```python
from build123d import *

# Parameters (mm, degrees)
SKETCH1_W                                          = 55
SKETCH1_H                                          = 24
BOSS_EXTRUDE1_DEPTH                                = 10
HOLE_WIZARD_3_D                                    = 4.5
HOLE_WIZARD_3_DEPTH                                = 12.4
HOLE_WIZARD_3_CBORE_D                              = 8
HOLE_WIZARD_3_CBORE_DEPTH                          = 4.6
HOLE_WIZARD_3_TIP                                  = 1.351936393
SKETCH6_W                                          = 5
SKETCH6_H                                          = 24
BOSS_EXTRUDE2_DEPTH                                = 10
CHAMFER1_SIZE                                      = 3
CHAMFER2_SIZE                                      = 0.5
HOLE_SIZE_BASED_ON_SOCKET_HEAD_CAP_SCR_D           = 5.5
HOLE_SIZE_BASED_ON_SOCKET_HEAD_CAP_SCR_DEPTH       = 12.4
HOLE_SIZE_BASED_ON_SOCKET_HEAD_CAP_SCR_CBORE_D     = 10
HOLE_SIZE_BASED_ON_SOCKET_HEAD_CAP_SCR_CBORE_DEPTH = 5.7
HOLE_SIZE_BASED_ON_SOCKET_HEAD_CAP_SCR_TIP         = 1.652366702
M5_TAPPED_HOLE1_D                                  = 4.2


with BuildPart() as part:
    # Sketch1 → Boss-Extrude1 (new body)
    with BuildSketch(Plane(origin=(0, 0, 0), x_dir=(1, 0, 0), z_dir=(0, 1, 0))):
        with Locations((-1.42708605, -3.163732927)):
            Rectangle(SKETCH1_W, SKETCH1_H)
    extrude(amount=BOSS_EXTRUDE1_DEPTH)

    # 打孔尺寸(%根据)内六角圆柱头螺钉的类型3
    with Locations(Plane(origin=(0, 0, 0), x_dir=(-1, 0, 0), z_dir=(0, -1, 0))):
        with Locations((23.92708605, -3.163732927), (-1.07291395, -3.163732927)):
            CounterBoreHole(HOLE_WIZARD_3_D / 2, HOLE_WIZARD_3_CBORE_D / 2, HOLE_WIZARD_3_CBORE_DEPTH, depth=HOLE_WIZARD_3_DEPTH)
            with Locations((0, 0, -(HOLE_WIZARD_3_DEPTH + HOLE_WIZARD_3_TIP / 2))):  # 118° drill point
                Cone(0, HOLE_WIZARD_3_D / 2, HOLE_WIZARD_3_TIP, mode=Mode.SUBTRACT)

    # Sketch6 → Boss-Extrude2 (add)
    with BuildSketch(Plane.XZ):
        with Locations((28.57291395, 3.163732927)):
            Rectangle(SKETCH6_W, SKETCH6_H)
    extrude(amount=-BOSS_EXTRUDE2_DEPTH)

    # Chamfer1
    chamfer1_edges = [part.edges().sort_by_distance(p)[0] for p in [
        (31.07291395, 5, 15.163732927),
        (31.07291395, 5, -8.836267073),
        (-28.92708605, 5, -8.836267073),
        (-28.92708605, 5, 15.163732927),
    ]]
    chamfer(chamfer1_edges, length=CHAMFER1_SIZE)

    # Chamfer2
    chamfer2_edges = [part.edges().sort_by_distance(p)[0] for p in [
        (1.07291395, 0, -8.836267073),
        (1.07291395, 10, -8.836267073),
        (-28.92708605, 0, 3.163732927),
        (31.07291395, 0, 3.163732927),
        (1.07291395, 0, 15.163732927),
        (31.07291395, 10, 3.163732927),
        (-28.92708605, 10, 3.163732927),
        (1.07291395, 10, 15.163732927),
    ]]
    chamfer(chamfer2_edges, length=CHAMFER2_SIZE)

    # Hole Size _Based On_ Socket Head Cap Scr
    with Locations(Plane(origin=(0, 0, 0), x_dir=(-1, 0, 0), z_dir=(0, -1, 0))):
        with Locations((-23.07291395, -3.163732927)):
            CounterBoreHole(HOLE_SIZE_BASED_ON_SOCKET_HEAD_CAP_SCR_D / 2, HOLE_SIZE_BASED_ON_SOCKET_HEAD_CAP_SCR_CBORE_D / 2, HOLE_SIZE_BASED_ON_SOCKET_HEAD_CAP_SCR_CBORE_DEPTH, depth=HOLE_SIZE_BASED_ON_SOCKET_HEAD_CAP_SCR_DEPTH)
            with Locations((0, 0, -(HOLE_SIZE_BASED_ON_SOCKET_HEAD_CAP_SCR_DEPTH + HOLE_SIZE_BASED_ON_SOCKET_HEAD_CAP_SCR_TIP / 2))):  # 118° drill point
                Cone(0, HOLE_SIZE_BASED_ON_SOCKET_HEAD_CAP_SCR_D / 2, HOLE_SIZE_BASED_ON_SOCKET_HEAD_CAP_SCR_TIP, mode=Mode.SUBTRACT)

    # M5 Tapped Hole1 (through all)
    with Locations(Plane(origin=(0, 10, 0), x_dir=(1, 0, 0), z_dir=(0, 1, 0))):
        with Locations((-11.92708605, -3.163732927), (13.07291395, -3.163732927)):
            Hole(M5_TAPPED_HOLE1_D / 2)


solid = part.part
```
Source: CAD feature listing. Evaluate the final solid. Frame: model axes, mm. A direction names the side the tool comes from. Coordinates: 2 decimals unless noted, no trailing zeros. Loops run counter-clockwise (first coordinate to the right, second up) from the corner with the lowest first, then second, coordinate; pieces in that order, holes last. Notation, with made-up numbers: (71, -12) -> (76, -12) arc R24 ccw to (76, 2) -> close; hole circle Ø2 at (-17.5, 16). An arc over 180 degrees is marked (long way). One line per item, written item: value. Start each with the question number.
Q1. Section query C-C, the plane x = -22.5. Return the cut outline in (y, z).
Q2. Contact query for flat-ended pins moving along their axis: P1, Ø7, axis at x = 1.07, z = 3.16, coming from the -Y side; P2, Ø6.5, axis at x = -23, z = 4.5, coming from the -Y side; P3, Ø9, axis at x = 23.07, z = 3.16, coming from the -Y side. Output: stop coordinate, or through.
Q3. Section query A-A, the plane x = 0.5. Return the cut outline in (y, z).
Q4. Section query D-D, the plane z = 4. Give the number of separate pieces and of enclosed holes in the cut face, and give its area (3 significant figures).
Q5. Set-up query: faces 5 (the face through (20.9, 5.7, 5.3)), 6 (the face through (0.78, 7.338, 0.933)). Return all of +Z, -Z, +X, -X, +Y, -Y with unobstructed straight access to the full face (end or side cutting, diameter ignored); none if empty.
Q6. Section query B-B, the plane y = 8.5. Return the cut outline in (x, z), and give its area (3 significant figures).
Q7. Mould query, pull axis Z, two halves, no side actions, for faces 1 (the face through (-27.448, 4.93, -7.315)), 2 (the face through (25.696, 7.88, 2.338)), 3 (the face through (5.07, 2.27, 2.99)), 4 (the face through (-27.45, 4.93, 13.64)). Classes: pulls with the +Z half, pulls with the -Z half, needs draft (parallel to the pull), parting line crosses it, or undercut.
Q8. Line query: line 1 along X through (y, z) = (4.5, -0.25); line 2 along X through (y, z) = (6.75, 4); line 3 along Z through (x, y) = (12, 3.5). Output: solid intervals per line, ascending.
Results:
1. outline: (0, -8.34) -> (0.5, -8.84) -> (9.5, -8.84) -> (10, -8.34) -> (10, 1.42) -> (4.6, 1.42) -> (4.6, -0.57) -> (0, -0.57) -> close; (0, 6.9) -> (4.6, 6.9) -> (4.6, 4.9) -> (10, 4.9) -> (10, 14.66) -> (9.5, 15.16) -> (0.5, 15.16) -> (0, 14.66) -> close
2. P1: y = 4.6
2. P2: y = 0
2. P3: y = 5.7
3. outline: (0, -8.34) -> (0.5, -8.84) -> (9.5, -8.84) -> (10, -8.34) -> (10, 0.99) -> (4.6, 0.99) -> (4.6, -0.8) -> (0, -0.8) -> close; (0, 7.12) -> (4.6, 7.12) -> (4.6, 5.34) -> (10, 5.34) -> (10, 14.66) -> (9.5, 15.16) -> (0.5, 15.16) -> (0, 14.66) -> close
4. separate pieces: 6
4. enclosed holes: 0
4. area: 327 mm^2
5. face 5: -Y
5. face 6: +Y, -Y
6. outline: (-28.93, -5.84) -> (-25.93, -8.84) -> (28.07, -8.84) -> (31.07, -5.84) -> (31.07, 12.16) -> (28.07, 15.16) -> (-25.93, 15.16) -> (-28.93, 12.16) -> close; hole circle Ø4.5 at (-23.93, 3.16); hole circle Ø4.2 at (-11.93, 3.16); hole circle Ø4.5 at (1.07, 3.16); hole circle Ø4.2 at (13.07, 3.16); hole circle Ø5.5 at (23.07, 3.16)
6. area: 1,340 mm^2
7. face 1: pulls with the -Z half
7. face 2: undercut
7. face 3: undercut
7. face 4: pulls with the +Z half
8. line 1: -28.93 to -26.01, -21.84 to -1.01, 3.16 to 19.42, 26.73 to 31.07
8. line 2: -28.93 to -26.02, -21.84 to -13.85, -10 to -1.02, 3.16 to 11.15, 15 to 20.45, 25.69 to 31.07
8. line 3: -8.84 to 1.36, 4.97 to 15.16
